Geometry: final body of the model. Coordinates: model frame, mm. A direction names the side the tool comes from. Give positions to 0.01 mm unless a question says otherwise; leave off trailing zeros. Loops run counter-clockwise (first coordinate to the right, second up) from the corner with the lowest first, then second, coordinate; pieces in that order, holes last.
from build123d import *

# Parameters (mm, degrees)
SKETCH1_W           = 12
SKETCH1_H           = 25
BOSS_EXTRUDE1_DEPTH = 3
SKETCH2_W           = 12
SKETCH2_H           = 15
BOSS_EXTRUDE2_DEPTH = 3
SKETCH3_R           = 2.5
BOSS_EXTRUDE3_DEPTH = 5
SCALE1_SCALE        = 2.5


with BuildPart() as part:
    # Sketch1 → Boss-Extrude1 (new body)
    with BuildSketch(Plane.XY):
        Rectangle(SKETCH1_W, SKETCH1_H)
    extrude(amount=BOSS_EXTRUDE1_DEPTH)

    # Sketch2 → Boss-Extrude2 (add)
    with BuildSketch(Plane.XY.offset(3)):
        Rectangle(SKETCH2_W, SKETCH2_H)
    extrude(amount=BOSS_EXTRUDE2_DEPTH)

    # Sketch3 → Boss-Extrude3 (add)
    with BuildSketch(Plane.XY.offset(6)):
        Circle(SKETCH3_R)
    extrude(amount=BOSS_EXTRUDE3_DEPTH)

    # Sketch4 → Revolve1 (revolve)
    with BuildSketch(Plane(origin=(0, 0, 0), x_dir=(1, 0, 0), z_dir=(0, 1, 0))):
        with BuildLine():
            Line((0, -11), (3, -11))
            ThreePointArc((3, -11), (2.121320344, -13.121320344), (0, -14))
            Line((0, -14), (0, -11))
        make_face()
    revolve(axis=Axis((0, 0, 11), (0, 0, 1)))


with BuildPart() as part_1:
    # Scale1: scaled about (0, 0, 0)
    add(part.part.scale(SCALE1_SCALE))


solid = part_1.part
Item 1: Set-up query: faces 4 (the face through (5.96, 1.88, 21.16)), 5 (the face through (0, 18.75, 11)), 6 (the face through (0, -18.75, 11)), 7 (the face through (0, -31.25, 4)). Return all of +Z, -Z, +X, -X, +Y, -Y with unobstructed straight access to the full face (end or side cutting, diameter ignored); none if empty.
Values follow:
face 4: none
face 5: +Z, +X, -X, +Y
face 6: +Z, +X, -X, -Y
face 7: +Z, -Z, +X, -X, -Y
Item 2: Section query B-B on y = 0. Return loops of the section in (x, z).
Values follow:
outline: (-15, 0) - (15, 0) - (15, 15) - (6.25, 15) - (6.25, 27.5) - (7.5, 27.5) arc R7.5 ccw to (-7.5, 27.5) - (-6.25, 27.5) - (-6.25, 15) - (-15, 15) - close
Item 3: Section query C-C on z = 25.5. Return loops of the section in (x, y).
Values follow:
outline: circle Ø12.5 at (0, 0)
Item 4: Ray query, probe 1 along Y at (x, z) = (-7.25, 11.5); probe 2 along Z at (x, y) = (-8.5, 1); probe 3 along Z at (x, y) = (9.25, 24.5). Return the intervals inside material, ascending.
Values follow:
probe 1: y = -18.75 to 18.75
probe 2: z = 0 to 15
probe 3: z = 0 to 7.5
Item 5: Pin query (flat end, axial travel): pin 1 (2 mm diameter, centred on x = -1, y = 6.5, fed in from +Z); pin 2 (12 mm diameter, centred on x = -7.5, z = 19.5, fed in from +Y); pin 3 (4 mm diameter, centred on x = -3, y = 22, fed in from +Z). Return the tip coordinate at first contact, or that it passes through.
Values follow:
pin 1: stops at z = 32.52
pin 2: stops at y = 18.75
pin 3: stops at z = 7.5
Item 6: Section query A-A on x = 0. Return loops of the section in (y, z), plus the area to 3 significant figures.
Values follow:
outline: (-31.25, 0) - (31.25, 0) - (31.25, 7.5) - (18.75, 7.5) - (18.75, 15) - (6.25, 15) - (6.25, 27.5) - (7.5, 27.5) arc R7.5 ccw to (-7.5, 27.5) - (-6.25, 27.5) - (-6.25, 15) - (-18.75, 15) - (-18.75, 7.5) - (-31.25, 7.5) - close
area: 995 mm2
Item 7: Section query D-D on x = 13.25. Return loops of the section in (y, z), plus the area to 3 significant figures.
Values follow:
outline: (-31.25, 0) - (31.25, 0) - (31.25, 7.5) - (18.75, 7.5) - (18.75, 15) - (-18.75, 15) - (-18.75, 7.5) - (-31.25, 7.5) - close
area: 750 mm2
Item 8: Draft query along Z for faces 1 (the face through (0, 25, 7.5)), 2 (the face through (0, 31.25, 4)), 3 (the face through (3, 6, 27.5)). Return one class per face: +Z half, -Z half, draft (parallel to the pull), parting line (faces both ways), or undercut.
Values follow:
face 1: +Z half
face 2: draft
face 3: undercut
